Answer from the drawing. Dimensions are ordinates in mm from the lowest x, y and z of the part. A direction names the side the tool comes from. Round coordinates to 2 decimals unless told otherwise and drop trailing zeros. Order: outer loops, then holes, each group sorted by start corner. A loop starts at its lowest first (then second) coordinate and runs counter-clockwise, first axis right, second up. Notation, with made-up numbers: (11, 17.5) -> (68, 17.5) arc R18 ccw to (68, 46.5) -> close; hole circle Ø7 at (33, -2). An arc over 180 degrees is marked (long way). Use a Markdown table: item, result. Add a question column.
1. Section A-A, the plane z = 32.5 is taken. Give the vertices of the cut face in (x, y), then the cut area to 3 significant figures.
2. Section D-D, the plane x = 42.5 is taken. Give the vertices of the cut face in (y, z).
3. For the marked faces 1 and 2, determine the directions among +Z, -Z, +X, -X, +Y, -Y from which every point of the face is accessible in a straight line to the end or side of a thin tool.
4. Consider L1, parallel to Z at x = 25, y = 3.75; L2, parallel to X at y = 8.75, z = 24.5; L3, parallel to Y at x = 42.5, z = 4. Determine where each line is inside the solid, lowest interval first. Write a range as [from, to].
5. Section B-B, the plane x = 25 is taken. Give the vertices of the cut face in (y, z).
6. Given pin 1 (6 mm diameter, centred on x = 7.5, y = 6, fed in from -Z), flat-ended and moving along its own axis, determine where the tip first touches the part or whether it passes through.
7. Section C-C, the plane y = 10.25 is taken. Give the vertices of the cut face in (x, z).
8. The mould has two halves that part along Y. Classify the marked faces 3, 4 and 5: +Y half, -Y half, draft (parallel to the pull), parting line (faces both ways), or undercut.
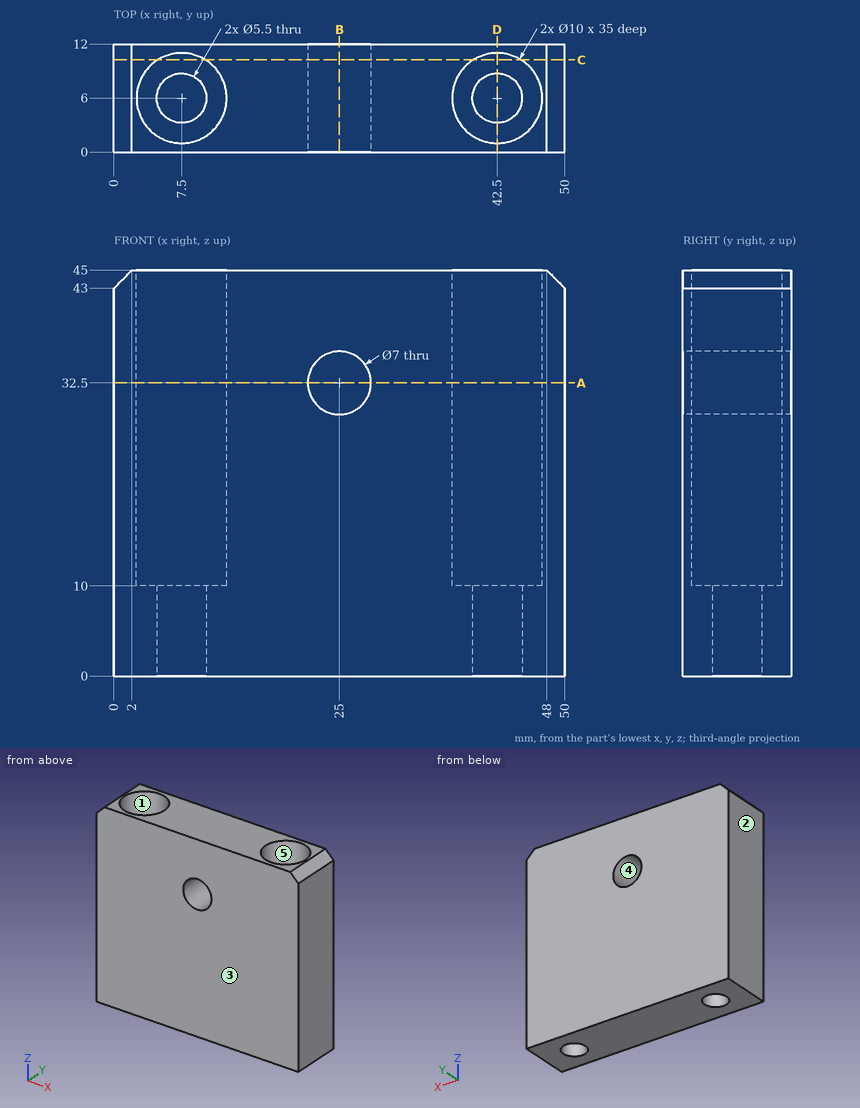
Verdict:
| question | item | result |
|---|---|---|
| 1 | outline | (0, 0) -> (21.5, 0) -> (21.5, 12) -> (0, 12) -> close; (28.5, 0) -> (50, 0) -> (50, 12) -> (28.5, 12) -> close; hole circle Ø10 at (7.5, 6); hole circle Ø10 at (42.5, 6) |
| 1 | area | 359 mm2 |
| 2 | outline | (0, 0) -> (3.25, 0) -> (3.25, 10) -> (1, 10) -> (1, 45) -> (0, 45) -> close; (8.75, 0) -> (12, 0) -> (12, 45) -> (11, 45) -> (11, 10) -> (8.75, 10) -> close |
| 3 | face 1 | +Z |
| 3 | face 2 | +Z, -Z, -X, +Y, -Y |
| 4 | L1 | z = [0, 29], [36, 45] |
| 4 | L2 | x = [0, 3.32], [11.68, 38.32], [46.68, 50] |
| 4 | L3 | y = [0, 3.25], [8.75, 12] |
| 5 | outline | (0, 0) -> (12, 0) -> (12, 29) -> (0, 29) -> close; (0, 36) -> (12, 36) -> (12, 45) -> (0, 45) -> close |
| 6 | pin 1 | stops at z = 0 |
| 7 | outline | (0, 0) -> (50, 0) -> (50, 43) -> (48, 45) -> (45.13, 45) -> (45.13, 10) -> (39.87, 10) -> (39.87, 45) -> (10.13, 45) -> (10.13, 10) -> (4.87, 10) -> (4.87, 45) -> (2, 45) -> (0, 43) -> close; hole circle Ø7 at (25, 32.5) |
| 8 | face 3 | -Y half |
| 8 | face 4 | draft |
| 8 | face 5 | undercut |
